Source: CAD feature listing. Evaluate the final solid. Frame: model axes, mm. A direction names the side the tool comes from. Give positions to 0.01 mm unless a question says otherwise; leave off trailing zeros. Order: outer loops, then holes, each group sorted by start corner. A loop starts at its lowest first (then second) coordinate and runs counter-clockwise, first axis right, second up. Notation, with made-up numbers: M 50,-10 L 63,-10 A25 cw 63,10 Z; hole C -9,0 d5. An arc over 180 degrees is marked long. Return JSON: item names as keys, results as strings.
from build123d import *

# Parameters (mm, degrees)
BOSS_EXTRUDE1_DEPTH = 6
SKETCH2_R           = 3
BOSS_EXTRUDE2_DEPTH = 65


with BuildPart() as part:
    # Sketch1 → Boss-Extrude1 (new body)
    with BuildSketch(Plane(origin=(0, 0, 0), x_dir=(1, 0, 0), z_dir=(0, 1, 0))):
        Polygon((-6.879699248, 12.868308957), (3.120300752, 12.868308957), (3.120300752, 14.668308957), (0.420300752, 17.368308957), (-4.179699248, 17.368308957), (-6.879699248, 14.668308957), align=None)
    extrude(amount=BOSS_EXTRUDE1_DEPTH)

    # Sketch2 → Boss-Extrude2 (add)
    with BuildSketch(Plane.XY.offset(-12.868308957)):
        with Locations(Location((-1.879699248, 3, 0), (0, 0, 270))):
            Circle(SKETCH2_R)
    extrude(amount=BOSS_EXTRUDE2_DEPTH)


solid = part.part
1. Ray query, probe 1 along Y at (x, z) = (-2, 25); probe 2 along X at (y, z) = (3.2, 45.5); probe 3 along Y at (x, z) = (-4.25, 24). Return the intervals inside material, ascending.
Evaluation:
{"probe 1": "y = 0 to 6", "probe 2": "x = -4.87 to 1.11", "probe 3": "y = 1.16 to 4.84"}
2. Section query B-B (x = -0.25). Return loops of the section in (y, z).
Evaluation:
{"outline": "M 0,-17.37 L 6,-17.37 L 6,-12.87 L 5.52,-12.87 L 5.52,52.13 L 0.48,52.13 L 0.48,-12.87 L 0,-12.87 Z"}
3. Section query D-D (x = -5.5). Return loops of the section in (y, z), then the cut area to 3 significant figures.
Evaluation:
{"outline": "M 0,-16.05 L 6,-16.05 L 6,-12.87 L 0,-12.87 Z", "area": "19.1 mm^2"}
4. Section query C-C (z = 11). Return loops of the section in (x, y), then the cut area to 3 significant figures.
Evaluation:
{"outline": "C -1.88,3 d6", "area": "28.3 mm^2"}
5. Set-up query: faces 1 (the face through (-2, 3, 52.132)), 2 (the face through (-4.81, 3.65, 19.18)). Return all of +Z, -Z, +X, -X, +Y, -Y with unobstructed straight access to the full face (end or side cutting, diameter ignored); none if empty.
Evaluation:
{"face 1": "+Z, +X, -X, +Y, -Y", "face 2": "+Z"}
6. First-contact query: pin 1 (1.5 mm diameter, centred on x = 0.5, z = 0, fed in from -Y); pin 2 (4 mm diameter, centred on x = 0.5, z = 39.5, fed in from -Y); pin 3 (5 mm diameter, centred on x = -5.5, z = 19, fed in from -Y). Flat tips, straight axial feed; report the tip coordinate or a pass-through.
Evaluation:
{"pin 1": "stops at y = 0.48", "pin 2": "stops at y = 0.02", "pin 3": "stops at y = 0.22"}
7. Section query A-A (y = 3). Return loops of the section in (x, z), then the cut area to 3 significant figures.
Evaluation:
{"outline": "M -6.88,-14.67 L -4.18,-17.37 L 0.42,-17.37 L 3.12,-14.67 L 3.12,-12.87 L 1.12,-12.87 L 1.12,52.13 L -4.88,52.13 L -4.88,-12.87 L -6.88,-12.87 Z", "area": "428 mm^2"}
